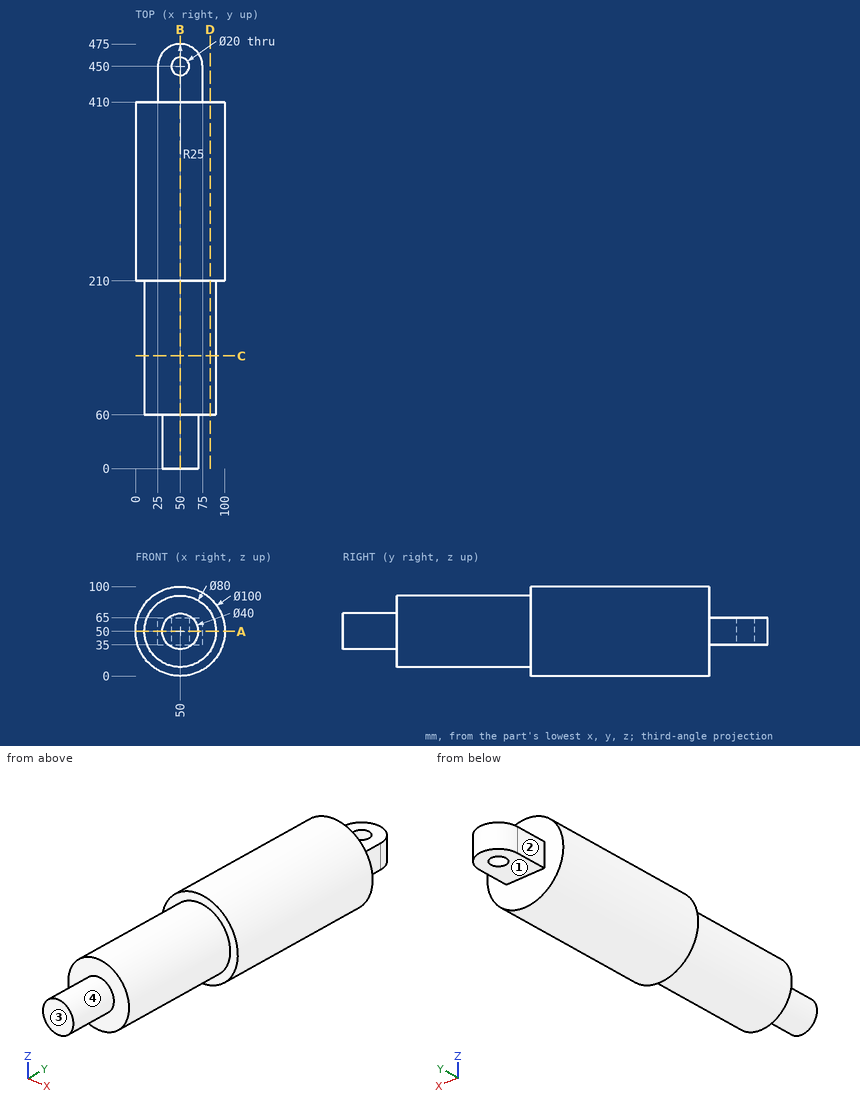
Design review of the part shown in the three views and the two pictorial views. Dimensions are in mm from the part's minimum x, y and z. A direction names the side the tool comes from. Give positions to 0.01 mm unless a question says otherwise; leave off trailing zeros. Write each loop counter-clockwise with the first axis right and the second up, starting at its lowest first coordinate (ties: lowest second). Pieces come first, ordered by that corner, then holes.
(1) Tool access review of the marked faces 1, 2, 3 and 4: name each direction out of +Z, -Z, +X, -X, +Y, -Y from which nothing blocks a thin tool from reaching the whole face with its end or side.
Checked values:
face 1: -Z, +X, -X, +Y
face 2: +Z, -Z, -X, +Y
face 3: +Z, -Z, +X, -X, -Y
face 4: -Y
(2) Clearance check with flat-ended pins moving along their axes: pin 1 Ø4 at (x, z) = (50, 79.5) entering from +Y; pin 2 Ø15 at (y, z) = (430.5, 49.5) entering from -X; pin 3 Ø12 at (y, z) = (138, 19) entering from +X (3 decimals); pin 4 Ø16 at (x, y) = (50, 450) entering from -Z. State where each tip first meets the part, or that it passes through.
Checked values:
pin 1: stops at y = 410
pin 2: stops at x = 25
pin 3: stops at x = 81.225
pin 4: passes through
(3) Add section A-A (z = 50). Give the boundary of the cut face in (x, y), and give its area (3 significant figures).
Checked values:
outline: (0, 210) - (10, 210) - (10, 60) - (30, 60) - (30, 0) - (70, 0) - (70, 60) - (90, 60) - (90, 210) - (100, 210) - (100, 410) - (75, 410) - (75, 450) arc R25 ccw to (25, 450) - (25, 410) - (0, 410) - close; hole circle Ø20 at (50, 450)
area: 37,100 mm2
(4) Wall thickness on line 1 along Y through (x, z) = (50, 55.25); line 2 along Y through (x, z) = (85.5, 25); line 3 along Y through (x, z) = (45, 70): over which ranges is each line inside the solid? List them lowest first.
Checked values:
line 1: y = 0 to 440, 460 to 475
line 2: y = 210 to 410
line 3: y = 60 to 410
(5) Add section B-B (x = 50). Give the boundary of the cut face in (y, z), and give its area (4 significant figures).
Checked values:
outline: (0, 30) - (60, 30) - (60, 10) - (210, 10) - (210, 0) - (410, 0) - (410, 35) - (440, 35) - (440, 65) - (410, 65) - (410, 100) - (210, 100) - (210, 90) - (60, 90) - (60, 70) - (0, 70) - close; (460, 35) - (475, 35) - (475, 65) - (460, 65) - close
area: 35,750 mm2
(6) Add section D-D (x = 83.5). Give the boundary of the cut face in (y, z).
Checked values:
outline: (60, 28.14) - (210, 28.14) - (210, 12.88) - (410, 12.88) - (410, 87.12) - (210, 87.12) - (210, 71.86) - (60, 71.86) - close
(7) Add section C-C (y = 126). Give the boundary of the cut face in (x, z), and give its area (3 significant figures).
Checked values:
outline: circle Ø80 at (50, 50)
area: 5,030 mm2
